Geometry check sheet. Reference: the model listing, model coordinates, mm. Face numbers are marked on the shaded views. A direction names the side the tool comes from. Coordinates: 2 decimals unless noted, no trailing zeros. Write each loop counter-clockwise with the first axis right and the second up, starting at its lowest first coordinate (ties: lowest second). Pieces come first, ordered by that corner, then holes. Notation, with made-up numbers: (38, 84.25) -> (51, 84.25) arc R14 cw to (51, 88.25) -> close; hole circle Ø3 at (56.5, 31). An arc over 180 degrees is marked (long way). Answer in a Markdown table with one row per item. Add a question column.
1. Cross-section at C-C on z = -8. Record the cut outline in (x, y).
2. Mould release check, pull along Y, two halves, no side actions. Record for the marked faces 5, 6 and 7: pulls with the +Y half, pulls with the -Y half, needs draft (parallel to the pull), parting line crosses it, or undercut.
3. Cross-section at A-A on y = 0. Record the cut outline in (x, z).
4. Cross-section at D-D on x = 25. Record the cut outline in (y, z), and give its area (3 significant figures).
5. Cross-section at B-B on x = 19. Record the cut outline in (y, z).
6. Depth check by flat-ended pin: P1, Ø7, axis at x = 44.5, z = -27.5, coming from the +Y side; P2, Ø0.5, axis at x = 43.5, z = 14, coming from the -Y side; P3, Ø2, axis at y = -3.5, z = -3, coming from the +X side. Enter the tip coordinate at first touch or a pass-through.
7. Set-up check for the marked faces 1, 2, 3 and 4: record each of +Z, -Z, +X, -X, +Y, -Y from which the full face is reachable in a straight line by a thin tool's end or side.
8. Scan lines: L1, parallel to Y at x = 19, z = -14.5; L2, parallel to X at y = 5, z = 17; L3, parallel to X at y = -12.5, z = 18. Record each from-to range of solid material in increasing order. Write a range as from..to.
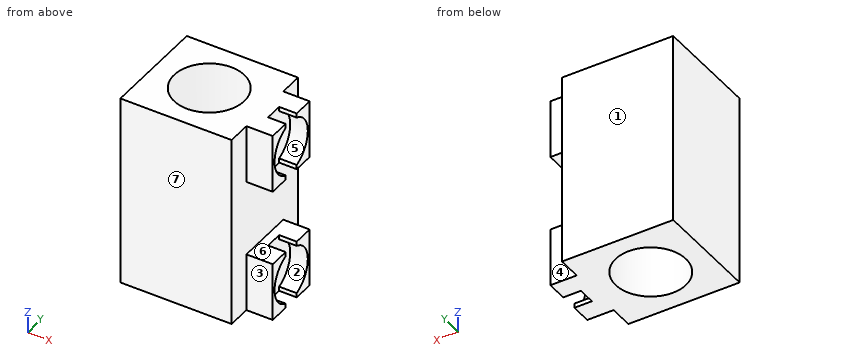
```python
from build123d import *

# Parameters (mm, degrees)
MAIN_BLOCK_PROFILE_W      = 66
MAIN_BLOCK_PROFILE_H      = 36
MAIN_BLOCK_66X36X38_DEPTH = 38
CLAMP_BOSSES_PROFILE_W    = 20
CLAMP_BOSSES_PROFILE_H    = 20
CLAMP_BOSSES_DEPTH        = 9
SADDLE_CUT_18_A_PROFILE_R = 9
SADDLE_CUT_18_A_DEPTH     = 6
NOTCH_A_3X3_DEPTH         = 84
NOTCH_A_3X3_DEPTH_BACK    = 6
NOTCH_B_3X3_DEPTH         = 6
SADDLE_CUT_18_B_PROFILE_R = 9
SADDLE_CUT_18_B_DEPTH     = 6
NOTCH_C_3X3_DEPTH         = 6
NOTCH_D_PROFILE_W         = 6
NOTCH_D_PROFILE_H         = 6
NOTCH_D_DEPTH             = 6
END_BORE_24_PROFILE_R     = 12
END_BORE_24_DEPTH         = 84


with BuildPart() as part:
    # Main Block Profile → Main Block 66x36x38 (new body)
    with BuildSketch(Plane(origin=(0, 0, 0), x_dir=(0, 0, -1), z_dir=(1, 0, 0))):
        Rectangle(MAIN_BLOCK_PROFILE_W, MAIN_BLOCK_PROFILE_H)
    extrude(amount=MAIN_BLOCK_66X36X38_DEPTH)

    # Clamp Bosses Profile → Clamp Bosses (add)
    with BuildSketch(Plane(origin=(38, 0, 0), x_dir=(0, 0, -1), z_dir=(1, 0, 0))):
        with Locations((-23, 0)):
            Rectangle(CLAMP_BOSSES_PROFILE_W, CLAMP_BOSSES_PROFILE_H)
        with Locations((23, 0)):
            Rectangle(CLAMP_BOSSES_PROFILE_W, CLAMP_BOSSES_PROFILE_H)
    extrude(amount=CLAMP_BOSSES_DEPTH)

    # Saddle Cut Ø18 A Profile → Saddle Cut Ø18 A (cut)
    with BuildSketch(Plane(origin=(47, 0, 0), x_dir=(0, 0, -1), z_dir=(1, 0, 0))):
        with Locations((-23, 0)):
            Circle(SADDLE_CUT_18_A_PROFILE_R)
    extrude(amount=-SADDLE_CUT_18_A_DEPTH, mode=Mode.SUBTRACT)

    # Notch A Profile → Notch A 3x3 (cut, two sides: drawn at the far end of the back side and taken through both)
    with BuildSketch(Plane.XY.offset(33).offset(-NOTCH_A_3X3_DEPTH_BACK)):
        Polygon((41, 3), (41, 0), (41, -3), (47, -3), (47, 3), align=None)
    extrude(amount=NOTCH_A_3X3_DEPTH + NOTCH_A_3X3_DEPTH_BACK, mode=Mode.SUBTRACT)

    # Notch B Profile → Notch B 3x3 (cut)
    with BuildSketch(Plane(origin=(0, 0, 13), x_dir=(-1, 0, 0), z_dir=(0, 0, -1))):
        Polygon((-41, 0), (-41, 3), (-47, 3), (-47, -3), (-41, -3), align=None)
    extrude(amount=-NOTCH_B_3X3_DEPTH, mode=Mode.SUBTRACT)

    # Saddle Cut Ø18 B Profile → Saddle Cut Ø18 B (cut)
    with BuildSketch(Plane(origin=(47, 0, 0), x_dir=(0, 0, -1), z_dir=(1, 0, 0))):
        with Locations((23, 0)):
            Circle(SADDLE_CUT_18_B_PROFILE_R)
    extrude(amount=-SADDLE_CUT_18_B_DEPTH, mode=Mode.SUBTRACT)

    # Notch C Profile → Notch C 3x3 (cut)
    with BuildSketch(Plane(origin=(0, 0, -33), x_dir=(-1, 0, 0), z_dir=(0, 0, -1))):
        Polygon((-41, 0), (-41, 3), (-47, 3), (-47, -3), (-41, -3), align=None)
    extrude(amount=-NOTCH_C_3X3_DEPTH, mode=Mode.SUBTRACT)

    # Notch D Profile → Notch D (cut)
    with BuildSketch(Plane.XY.offset(-13)):
        with Locations((44, 0)):
            Rectangle(NOTCH_D_PROFILE_W, NOTCH_D_PROFILE_H)
    extrude(amount=-NOTCH_D_DEPTH, mode=Mode.SUBTRACT)

    # End Bore Ø24 Profile → End Bore Ø24 (cut, through all)
    with BuildSketch(Plane.XY.offset(33)):
        with Locations((19, 0)):
            Circle(END_BORE_24_PROFILE_R)
    extrude(amount=-END_BORE_24_DEPTH, mode=Mode.SUBTRACT)


solid = part.part
```
Results found:
| question | item | result |
|---|---|---|
| 1 | outline | (0, -18) -> (38, -18) -> (38, 18) -> (0, 18) -> close; hole circle Ø24 at (19, 0) |
| 2 | face 5 | undercut |
| 2 | face 6 | needs draft |
| 2 | face 7 | pulls with the -Y half |
| 3 | outline | (0, -33) -> (7, -33) -> (7, 33) -> (0, 33) -> close; (31, -33) -> (41, -33) -> (41, -13) -> (38, -13) -> (38, 13) -> (41, 13) -> (41, 33) -> (31, 33) -> close |
| 4 | outline | (-18, -33) -> (-10.39, -33) -> (-10.39, 33) -> (-18, 33) -> close; (10.39, -33) -> (18, -33) -> (18, 33) -> (10.39, 33) -> close |
| 4 | area | 1,000 mm^2 |
| 5 | outline | (-18, -33) -> (-12, -33) -> (-12, 33) -> (-18, 33) -> close; (12, -33) -> (18, -33) -> (18, 33) -> (12, 33) -> close |
| 6 | P1 | stops at y = 10 |
| 6 | P2 | stops at y = -10 |
| 6 | P3 | stops at x = 38 |
| 7 | face 1 | +Z, -Z, +X, -X, +Y |
| 7 | face 2 | +X |
| 7 | face 3 | +Z, -Z, +X, -Y |
| 7 | face 4 | +Z, -Z, +X, +Y |
| 8 | L1 | y = -18..-12, 12..18 |
| 8 | L2 | x = 0..8.09, 29.91..41 |
| 8 | L3 | x = 0..38 |
